```python
from build123d import *

# Parameters (mm, degrees)
SKETCH2_W          = 3.587001172
SKETCH2_H          = 15.298776085
CUT_EXTRUDE1_DEPTH = 12.8
SKETCH3_W          = 4.275598186
SKETCH3_H          = 2


with BuildPart() as part:
    # Sketch1 → Revolve1 (revolve)
    with BuildSketch(Plane.XY, mode=Mode.PRIVATE) as revolve1_sk:
        Polygon((0, 0), (7.5, 0), (7.5, 147.2), (5, 147.2), (5, 160), (4, 160), (4, 170), (0, 170), align=None)
    revolve(revolve1_sk.sketch.rotate(Axis((0, -11.254736842, 0), (0, 1, 0)), 90), axis=Axis((0, -11.254736842, 0), (0, 1, 0)))

    # Sketch2 → Cut-Extrude1 (cut)
    with BuildSketch(Plane(origin=(0, 160, 0), x_dir=(1, 0, 0), z_dir=(0, 1, 0))):
        with Locations((-6.293500586, -0.885946073)):
            Rectangle(SKETCH2_W, SKETCH2_H)
    extrude(amount=-CUT_EXTRUDE1_DEPTH, mode=Mode.SUBTRACT)

    # Sketch3 → Cut-Revolve1 (revolve, cut)
    with BuildSketch(Plane.XY, mode=Mode.PRIVATE) as cut_revolve1_sk:
        with Locations((8.137799093, 7)):
            Rectangle(SKETCH3_W, SKETCH3_H)
    revolve(cut_revolve1_sk.sketch.rotate(Axis((0, 0, 0), (0, 1, 0)), 90), axis=Axis((0, 0, 0), (0, 1, 0)), mode=Mode.SUBTRACT)


solid = part.part
```
Work out the finished part from the listing and answer in its coordinate system (mm). A direction names the side the tool comes from. Give positions to 0.01 mm unless a question says otherwise; leave off trailing zeros. Order: outer loops, then holes, each group sorted by start corner. A loop starts at its lowest first (then second) coordinate and runs counter-clockwise, first axis right, second up. Notation, with made-up numbers: (-3, -0.75) - (34, -0.75) arc R11 ccw to (34, 19.25) - close; hole circle Ø6 at (-29, 74.25). An arc over 180 degrees is marked (long way). One line per item, written item: value. Start each with the question number.
1. Each of these flat-tipped pins is pushed along its axis until it touches: pin 1 Ø8 at (x, z) = (1, -4.5) entering from +Y; pin 2 Ø5 at (y, z) = (54, 3) entering from -X; pin 3 Ø1.5 at (x, z) = (-3.5, -4.5) entering from +Y; pin 4 Ø5 at (y, z) = (152, -0.5) entering from -X. Where does it stop, or does it pass through?
2. For a pull along Y with two mould halves and no side action, classify faces 4 (the face through (0, 170, 0)), 5 (the face through (-6.324, 3.042, -4.032)), 6 (the face through (-1.802, 7.014, -5.723)) as released by +Y, released by -Y, zero draft, split by the parting line, or undercut.
3. Section C-C, the plane y = 11 is taken. Write down the section's boundary in (x, z).
4. Consider line 1 (Y direction, x = -5.75, z = -2.5); line 2 (X direction, y = 84, z = -0.25); line 3 (Y direction, x = -3, z = 3.5). Determine where each line is inside the solid, lowest interval first.
5. Section A-A, the plane z = 0 is taken. Write down the section's boundary in (x, y), then the cut area to 3 significant figures.
6. Section B-B, the plane x = 0 is taken. Write down the section's boundary in (y, z).
7. Which of the six approach directions +Z, -Z, +X, -X, +Y, -Y give full straight-line access (tool end or side, diameter ignored) to faces 1 (the face through (-6, 6, 2)), 2 (the face through (-4.5, 154, 0)), 3 (the face through (2, 147.2, -5))?
Filled sheet:
1. pin 1: y = 170
1. pin 2: x = -7.48
1. pin 3: y = 160
1. pin 4: x = -4.5
2. face 4: released by +Y
2. face 5: zero draft
2. face 6: undercut
3. outline: circle Ø15 at (0, 0)
4. line 1: 0 to 6, 8 to 147.2
4. line 2: -7.5 to 7.5
4. line 3: 0 to 160
5. outline: (-7.5, 0) - (7.5, 0) - (7.5, 6) - (6, 6) - (6, 8) - (7.5, 8) - (7.5, 147.2) - (5, 147.2) - (5, 160) - (4, 160) - (4, 170) - (-4, 170) - (-4, 160) - (-4.5, 160) - (-4.5, 147.2) - (-7.5, 147.2) - (-7.5, 8) - (-6, 8) - (-6, 6) - (-7.5, 6) - close
5. area: 2,400 mm²
6. outline: (0, -7.5) - (6, -7.5) - (6, -6) - (8, -6) - (8, -7.5) - (147.2, -7.5) - (147.2, -5) - (160, -5) - (160, -4) - (170, -4) - (170, 4) - (160, 4) - (160, 5) - (147.2, 5) - (147.2, 7.5) - (8, 7.5) - (8, 6) - (6, 6) - (6, 7.5) - (0, 7.5) - close
7. face 1: none
7. face 2: +Z, -Z, -X, +Y
7. face 3: +Y
